from build123d import *

# Parameters (mm, degrees)
SKETCH1_W                                           = 60
SKETCH1_H                                           = 170.4
BOSS_EXTRUDE1_DEPTH                                 = 6
CBORE_FOR_M5_HEX_SOCKET_HEAD_CAP_SCREW1_D           = 5.5
CBORE_FOR_M5_HEX_SOCKET_HEAD_CAP_SCREW1_CBORE_D     = 10
CBORE_FOR_M5_HEX_SOCKET_HEAD_CAP_SCREW1_CBORE_DEPTH = 5.4
BLIND_PIN_HOLE0_D                                   = 5
M4_TAPPED_HOLE1_D                                   = 3.3
SKETCH11_R                                          = 3.5
CUT_EXTRUDE1_DEPTH                                  = 2
M6_TAPPED_HOLE1_D                                   = 5
M6_TAPPED_HOLE1_DEPTH                               = 17
M6_TAPPED_HOLE1_TIP                                 = 1.502151548
CHAMFER1_SIZE                                       = 1
BLIND_PIN_HOLE1_D                                   = 4
M5_TAPPED_HOLE1_D                                   = 4.2


with BuildPart() as part:
    # Sketch1 → Boss-Extrude1 (new, symmetric)
    with BuildSketch(Plane.XY):
        Rectangle(SKETCH1_W, SKETCH1_H)
    extrude(amount=BOSS_EXTRUDE1_DEPTH, both=True)

    # CBORE for M5 Hex Socket Head Cap Screw1 (through all)
    with Locations(Plane(origin=(0, 0, -6), x_dir=(-1, 0, 0), z_dir=(0, 0, -1))):
        with Locations((15, -5.2), (-15, -5.2), (15, -79.2), (-15, -79.2)):
            CounterBoreHole(CBORE_FOR_M5_HEX_SOCKET_HEAD_CAP_SCREW1_D / 2, CBORE_FOR_M5_HEX_SOCKET_HEAD_CAP_SCREW1_CBORE_D / 2, CBORE_FOR_M5_HEX_SOCKET_HEAD_CAP_SCREW1_CBORE_DEPTH)

    # Blind pin hole0 (through all)
    with Locations(Plane.XY.offset(6)):
        with Locations((20, 3.3), (-20, 3.3)):
            Hole(BLIND_PIN_HOLE0_D / 2)

    # M4 Tapped Hole1 (through all)
    with Locations(Plane(origin=(0, 0, -6), x_dir=(-1, 0, 0), z_dir=(0, 0, -1))):
        with Locations((0, 11.7), (0, -28.3), (0, -48.3), (0, -68.3), (0, 51.7)):
            Hole(M4_TAPPED_HOLE1_D / 2)

    # Sketch11 → Cut-Extrude1 (cut)
    with BuildSketch(Plane(origin=(0, 0, -6), x_dir=(-1, 0, 0), z_dir=(0, 0, -1))):
        with Locations((0, 51.7)):
            Circle(SKETCH11_R)
        with Locations((0, -68.3)):
            Circle(SKETCH11_R)
    extrude(amount=-CUT_EXTRUDE1_DEPTH, mode=Mode.SUBTRACT)

    # M6 Tapped Hole1
    with Locations(Plane.XY.offset(6)):
        with Locations((8.5, 57.2), (-8.5, 57.2), (8.5, 71.2), (-8.5, 71.2)):
            Hole(M6_TAPPED_HOLE1_D / 2, depth=M6_TAPPED_HOLE1_DEPTH)
            with Locations((0, 0, -(M6_TAPPED_HOLE1_DEPTH + M6_TAPPED_HOLE1_TIP / 2))):  # 118° drill point
                Cone(0, M6_TAPPED_HOLE1_D / 2, M6_TAPPED_HOLE1_TIP, mode=Mode.SUBTRACT)

    # Chamfer1
    chamfer1_edges = [part.edges().sort_by_distance(p)[0] for p in [
        (30, -85.2, 0),
        (-30, -85.2, 0),
        (-30, 85.2, 0),
        (30, 85.2, 0),
    ]]
    chamfer(chamfer1_edges, length=CHAMFER1_SIZE)

    # Blind pin hole1 (through all)
    with Locations(Plane(origin=(0, 0, -6), x_dir=(-1, 0, 0), z_dir=(0, 0, -1))):
        with Locations((23.5, -36.8), (-23.5, -36.8)):
            Hole(BLIND_PIN_HOLE1_D / 2)

    # M5 Tapped Hole1 (through all)
    with Locations(Plane(origin=(0, 0, -6), x_dir=(-1, 0, 0), z_dir=(0, 0, -1))):
        with Locations((23.5, 62.2), (-23.5, -24.3), (-23.5, -49.3), (23.5, -49.3), (23.5, -24.3), (-23.5, 62.2)):
            Hole(M5_TAPPED_HOLE1_D / 2)


solid = part.part
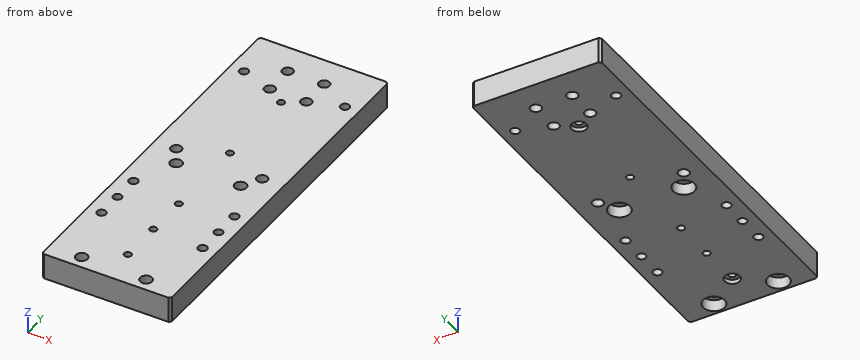
Model file for the job. Use its own axes, mm. Round coordinates to 2 decimals unless told otherwise and drop trailing zeros. Loops run counter-clockwise (first coordinate to the right, second up) from the corner with the lowest first, then second, coordinate; pieces in that order, holes last. Notation, with made-up numbers: (5, -9.5) - (24, -9.5) arc R28 cw to (24, 12.5) - close; hole circle Ø8 at (-23, 47.5). An arc over 180 degrees is marked (long way). Write each question's results on one line, items separated by ' | '.
(1) Saw through at C-C, the plane y = 62.2. List the corners of the cut face in (x, z), then the cut area to 3 significant figures.
Answer below:
outline: (-30, -6) - (-25.6, -6) - (-25.6, 6) - (-30, 6) - close; (-21.4, -6) - (21.4, -6) - (21.4, 6) - (-21.4, 6) - close; (25.6, -6) - (30, -6) - (30, 6) - (25.6, 6) - close | area: 619 mm^2
(2) Wall check: L1, parallel to Y at x = 8.5, z = 1.5; L2, parallel to Y at x = -15, z = -3.95; L3, parallel to Y at x = 0, z = 2.25. Give the ranges that are in metal, low to high.
Answer below:
L1: y = -85.2 to 54.7, 59.7 to 68.7, 73.7 to 85.2 | L2: y = -85.2 to -84.2, -74.2 to -10.2, -0.2 to 85.2 | L3: y = -85.2 to -69.95, -66.65 to -49.95, -46.65 to -29.95, -26.65 to 10.05, 13.35 to 50.05, 53.35 to 85.2
(3) Pin check, flat tips, straight feed: pin 1 (8 mm diameter, centred on x = 13, y = -7, fed in from -Z); pin 2 (5 mm diameter, centred on x = -14.5, y = -3, fed in from -Z). Stop position of each tip, or through.
Answer below:
pin 1: stops at z = -6 | pin 2: stops at z = -0.6
(4) Saw through at B-B, the plane z = 3. Count the separate pieces of the cut face and the enclosed holes in it, then the cut area to 3 significant figures.
Answer below:
separate pieces: 1 | enclosed holes: 23 | area: 9,860 mm^2
(5) Saw through at A-A, the plane x = 15. List the corners of the cut face in (y, z), then the cut area to 3 significant figures.
Answer below:
outline: (-85.2, -6) - (-84.2, -6) - (-84.2, -0.6) - (-81.95, -0.6) - (-81.95, 6) - (-85.2, 6) - close; (-76.45, -0.6) - (-74.2, -0.6) - (-74.2, -6) - (-10.2, -6) - (-10.2, -0.6) - (-7.95, -0.6) - (-7.95, 6) - (-76.45, 6) - close; (-2.45, -0.6) - (-0.2, -0.6) - (-0.2, -6) - (85.2, -6) - (85.2, 6) - (-2.45, 6) - close | area: 1,860 mm^2
